Read the model definition and answer for the solid it produces. Units are mm, in the model's axes. Round coordinates to 2 decimals unless told otherwise and drop trailing zeros. Write each loop counter-clockwise with the first axis right and the second up, starting at its lowest first coordinate (ties: lowest second). Pieces come first, ordered by that corner, then holes. Notation, with made-up numbers: (58.5, -7) -> (98.5, -7) arc R7 cw to (98.5, 2) -> close; hole circle Ø6 at (24.5, 86.25). An arc over 180 degrees is marked (long way). Return JSON: item names as keys, results as strings.
from build123d import *

# Parameters (mm, degrees)
SKETCH_1_R      = 4
SKETCH_1_R_2    = 10
EXTRUDE_1_DEPTH = 7


with BuildPart() as part:
    # 草图1 → 凸台-拉伸1 (new body)
    with BuildSketch(Plane(origin=(797.597549653, 0, 0), x_dir=(0, 0, -1), z_dir=(1, 0, 0))):
        with BuildLine():
            Line((-188.626135314, -11.329587329), (348.639550057, 21.957895527))
            ThreePointArc((348.639550057, 21.957895527), (371.957895527, 1.360449943), (351.360449943, -21.957895527))
            Line((351.360449943, -21.957895527), (-185.905235429, -55.245378382))
            ThreePointArc((-185.905235429, -55.245378382), (-209.223580898, -34.647932798), (-188.626135314, -11.329587329))
        make_face()
        with Locations(Location((350, 0, 0), (0, 0, 90))):
            Circle(SKETCH_1_R, mode=Mode.SUBTRACT)
        with Locations(Location((-187.265685371, -33.287482855, 0), (0, 0, 90))):
            Circle(SKETCH_1_R_2, mode=Mode.SUBTRACT)
    extrude(amount=-EXTRUDE_1_DEPTH)


solid = part.part
Item 1: Straight lines are drawn through the part: L1, parallel to Y at x = 795.5, z = -350; L2, parallel to Y at x = 791.5, z = 157; L3, parallel to Z at x = 795.25, y = -16. For each, find the intervals that lie inside material, in ascending order. Write a range as [from, to].
Worked answers:
{"L1": "y = [-22.04, -4], [4, 22]", "L2": "y = [-53.45, -9.37]", "L3": "z = [-365.1, 200.87]"}
Item 2: Section A-A (y = -30) is taken. Give the vertices of the cut face in (x, z).
Worked answers:
{"outline": "(790.6, -221.56) -> (797.6, -221.56) -> (797.6, 177.82) -> (790.6, 177.82) -> close; (790.6, 196.71) -> (797.6, 196.71) -> (797.6, 209.02) -> (790.6, 209.02) -> close"}
Item 3: For a pull along Y with two mould halves and no side action, classify faces 1 (the cylindrical face through (794.147, -35.455, 177.503)), 2 (the flat face through (790.598, -16, -85)), 3 (the flat face through (794.15, 5.08, -76.25)), 4 (the cylindrical face through (794.15, -35.13, 209.19)) as released by +Y, released by -Y, zero draft, split by the parting line, or undercut.
Worked answers:
{"face 1": "undercut", "face 2": "zero draft", "face 3": "released by +Y", "face 4": "split by the parting line"}
Item 4: Section C-C (z = -302.5) is taken. Give the vertices of the cut face in (x, y).
Worked answers:
{"outline": "(790.6, -24.99) -> (797.6, -24.99) -> (797.6, 19.1) -> (790.6, 19.1) -> close"}
Item 5: Section B-B (x = 796.5) is taken. Give the vertices of the cut face in (y, z).
Worked answers:
{"outline": "(-55.25, 185.91) -> (-21.96, -351.36) arc R22 ccw to (21.96, -348.64) -> (-11.33, 188.63) arc R22 ccw to start; hole circle Ø20 at (-33.29, 187.27); hole circle Ø8 at (0, -350)"}
Item 6: Flat-ended cylindrical pins translate along their axes: pin 1 (1 mm diameter, centred on x = 792, y = -5.5, fed in from -Z); pin 2 (3 mm diameter, centred on x = 794.5, z = -0.5, fed in from +Y); pin 3 (3 mm diameter, centred on x = 795, y = -15, fed in from +Z). Find the tip coordinate at first contact, or state that the pin passes through.
Worked answers:
{"pin 1": "stops at z = -371.42", "pin 2": "stops at y = 0.48", "pin 3": "stops at z = 201.48"}
